from build123d import *

# Parameters (mm, degrees)
EXTRUDE_1_DEPTH     = 32.5
CUT_EXTRUDE_1_REACH = 140.247
SKETCH_3_W          = 46
SKETCH_3_H          = 25
EXTRUDE_2_DEPTH     = 10


with BuildPart() as part:
    # 草图1 → 凸台-拉伸1 (new, symmetric)
    with BuildSketch(Plane.XY):
        Polygon((0, 0), (0, 34), (10, 34), (10, 10), (140, 10), (140, 0), align=None)
    extrude(amount=EXTRUDE_1_DEPTH, both=True)

    # 草图2 → 切除-拉伸1 (cut, up to next)
    with BuildSketch(Plane(origin=(10, 0, 0), x_dir=(0, 0, -1), z_dir=(1, 0, 0)), mode=Mode.PRIVATE) as cut_extrude_1_sk1:
        with BuildLine():
            Line((-26.5, 31), (-22.5, 31))
            ThreePointArc((-22.5, 31), (-19.5, 28), (-22.5, 25))
            Line((-22.5, 25), (-26.5, 25))
            ThreePointArc((-26.5, 25), (-29.5, 28), (-26.5, 31))
        make_face()
    cut_extrude_1_tool1 = extrude(cut_extrude_1_sk1.sketch, amount=-CUT_EXTRUDE_1_REACH, mode=Mode.PRIVATE) & part.part
    # 草图2 → 切除-拉伸1 (cut, up to next)
    with BuildSketch(Plane(origin=(10, 0, 0), x_dir=(0, 0, -1), z_dir=(1, 0, 0)), mode=Mode.PRIVATE) as cut_extrude_1_sk2:
        with BuildLine():
            Line((22.5, 31), (26.5, 31))
            ThreePointArc((26.5, 31), (29.5, 28), (26.5, 25))
            Line((26.5, 25), (22.5, 25))
            ThreePointArc((22.5, 25), (19.5, 28), (22.5, 31))
        make_face()
    cut_extrude_1_tool2 = extrude(cut_extrude_1_sk2.sketch, amount=-CUT_EXTRUDE_1_REACH, mode=Mode.PRIVATE) & part.part
    # 草图2 → 切除-拉伸1 (cut, up to next)
    with BuildSketch(Plane(origin=(10, 0, 0), x_dir=(0, 0, -1), z_dir=(1, 0, 0)), mode=Mode.PRIVATE) as cut_extrude_1_sk3:
        with BuildLine():
            Line((-26.5, 13), (-22.5, 13))
            ThreePointArc((-22.5, 13), (-19.5, 16), (-22.5, 19))
            Line((-22.5, 19), (-26.5, 19))
            ThreePointArc((-26.5, 19), (-29.5, 16), (-26.5, 13))
        make_face()
    cut_extrude_1_tool3 = extrude(cut_extrude_1_sk3.sketch, amount=-CUT_EXTRUDE_1_REACH, mode=Mode.PRIVATE) & part.part
    # 草图2 → 切除-拉伸1 (cut, up to next)
    with BuildSketch(Plane(origin=(10, 0, 0), x_dir=(0, 0, -1), z_dir=(1, 0, 0)), mode=Mode.PRIVATE) as cut_extrude_1_sk4:
        with BuildLine():
            Line((22.5, 13), (26.5, 13))
            ThreePointArc((26.5, 13), (29.5, 16), (26.5, 19))
            Line((26.5, 19), (22.5, 19))
            ThreePointArc((22.5, 19), (19.5, 16), (22.5, 13))
        make_face()
    cut_extrude_1_tool4 = extrude(cut_extrude_1_sk4.sketch, amount=-CUT_EXTRUDE_1_REACH, mode=Mode.PRIVATE) & part.part
    add(cut_extrude_1_tool1.solids().sort_by_distance((10, 28, 24.5))[0], mode=Mode.SUBTRACT)
    add(cut_extrude_1_tool2.solids().sort_by_distance((10, 28, -24.5))[0], mode=Mode.SUBTRACT)
    add(cut_extrude_1_tool3.solids().sort_by_distance((10, 16, 24.5))[0], mode=Mode.SUBTRACT)
    add(cut_extrude_1_tool4.solids().sort_by_distance((10, 16, -24.5))[0], mode=Mode.SUBTRACT)

    # 草图3 → 凸台-拉伸2 (add)
    with BuildSketch(Plane(origin=(0, 10, 0), x_dir=(1, 0, 0), z_dir=(0, 1, 0))):
        with Locations((117, -45)):
            Rectangle(SKETCH_3_W, SKETCH_3_H)
    extrude(amount=-EXTRUDE_2_DEPTH)


solid = part.part
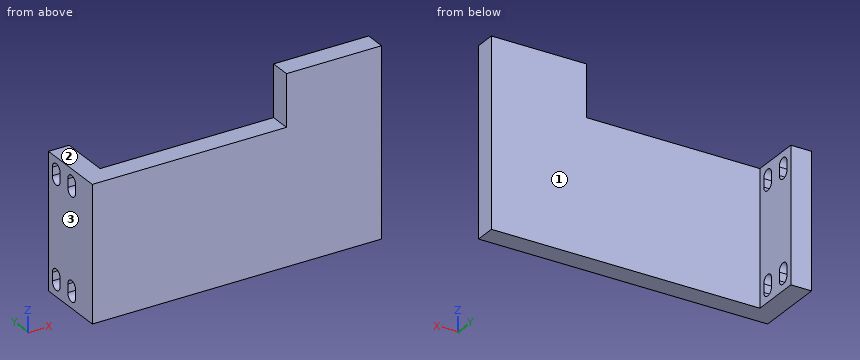
For this review, take the finished solid that the model builds, in its own axes (mm). Face numbers are marked on the shaded views. A direction names the side the tool comes from. Coordinates: 2 decimals unless noted, no trailing zeros. Order: outer loops, then holes, each group sorted by start corner. A loop starts at its lowest first (then second) coordinate and runs counter-clockwise, first axis right, second up. Notation, with made-up numbers: (36.25, -6) -> (92.25, -6) arc R22 cw to (92.25, 10) -> close; hole circle Ø3 at (54.5, 57.25). An arc over 180 degrees is marked (long way). Return JSON: item names as keys, results as strings.
1. We need section C-C on y = 17.5. Write out the cut boundary in (x, z).
Answer block:
{"outline": "(0, -32.5) -> (10, -32.5) -> (10, -29.1) -> (0, -29.1) -> close; (0, -19.9) -> (10, -19.9) -> (10, 19.9) -> (0, 19.9) -> close; (0, 29.1) -> (10, 29.1) -> (10, 32.5) -> (0, 32.5) -> close"}
2. We need section D-D on z = 37.5. Write out the cut boundary in (x, y).
Answer block:
{"outline": "(94, 0) -> (140, 0) -> (140, 10) -> (94, 10) -> close"}
3. We need section B-B on x = 44. Write out the cut boundary in (y, z), and give its area (3 significant figures).
Answer block:
{"outline": "(0, -32.5) -> (10, -32.5) -> (10, 32.5) -> (0, 32.5) -> close", "area": "650 mm²"}
4. For line 1 (X direction, y = 9, z = 38.5); line 2 (Y direction, x = 115.5, z = 20), list the stretches that pass through material, from the lowest coordinate up. Write a range as from..to.
Answer block:
{"line 1": "94..140", "line 2": "0..10"}
5. For pin 1 Ø1.5 at (x, z) = (63.5, 28.5) entering from +Y; pin 2 Ø7 at (y, z) = (25, -5) entering from +X; pin 3 Ø5 at (y, z) = (4.5, 41) entering from -X, all flat-tipped, find the tip position at first contact; note any pin that passes through.
Answer block:
{"pin 1": "y = 10", "pin 2": "x = 10", "pin 3": "x = 94"}
6. Machinability: for the marked faces 1, 2 and 3, which of the approach directions +Z, -Z, +X, -X, +Y, -Y give a long, thin tool a straight path to every point of the face, cutting with its end or side? Answer none if there is none.
Answer block:
{"face 1": "+Z, -Z, +X, +Y", "face 2": "+Z, -X, +Y, -Y", "face 3": "+Z, -Z, -X, +Y, -Y"}
7. We need section A-A on y = 28. Write out the cut boundary in (x, z), and give its area (3 significant figures).
Answer block:
{"outline": "(0, -32.5) -> (10, -32.5) -> (10, -29.5) -> (0, -29.5) -> close; (0, -19.5) -> (10, -19.5) -> (10, 19.5) -> (0, 19.5) -> close; (0, 29.5) -> (10, 29.5) -> (10, 32.5) -> (0, 32.5) -> close", "area": "450 mm²"}
